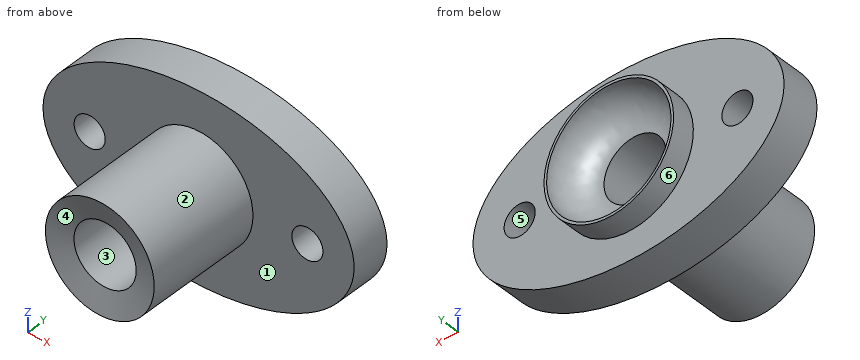
```python
from build123d import *

# Parameters (mm, degrees)
SHANK_SKETCH_42_R          = 21
SHANK_42_DEPTH             = 45
FLANGE_SKETCH_120X36_RX    = 60
FLANGE_SKETCH_120X36_RY    = 36
OVAL_FLANGE_120X36_DEPTH   = 15
SPIGOT_SKETCH_50_R         = 25
SPIGOT_50_DEPTH            = 9
MOUNTING_HOLES_SKETCH_R    = 6
MOUNTING_HOLES_2X_12_DEPTH = 19


with BuildPart() as part:
    # Shank Sketch Ø42 → Shank Ø42 (new body)
    with BuildSketch(Plane(origin=(0, 0, 0), x_dir=(1, 0, 0), z_dir=(0, 1, 0))):
        with Locations(Location((0, 0, 0), (0, 0, 90))):
            Circle(SHANK_SKETCH_42_R)
    extrude(amount=SHANK_42_DEPTH)

    # Flange Sketch 120x36 → Oval Flange 120x36 (add)
    with BuildSketch(Plane(origin=(0, 45, 0), x_dir=(1, 0, 0), z_dir=(0, 1, 0))):
        with Locations((0, 0)):
            Ellipse(FLANGE_SKETCH_120X36_RX, FLANGE_SKETCH_120X36_RY)
    extrude(amount=OVAL_FLANGE_120X36_DEPTH)

    # Spigot Sketch Ø50 → Spigot Ø50 (add)
    with BuildSketch(Plane(origin=(0, 60, 0), x_dir=(1, 0, 0), z_dir=(0, 1, 0))):
        with Locations(Location((0, 0, 0), (0, 0, 270))):
            Circle(SPIGOT_SKETCH_50_R)
    extrude(amount=SPIGOT_50_DEPTH)

    # Bore Profile Sketch → Bore and Seat Cut (revolve, cut)
    with BuildSketch(Plane.XY, mode=Mode.PRIVATE) as bore_and_seat_cut_sk:
        with BuildLine():
            Line((21, 0), (12, 2.411542732))
            Line((12, 2.411542732), (12, 57))
            ThreePointArc((12, 57), (20.485281374, 60.514718626), (24, 69))
            Line((24, 69), (0, 69))
            Line((0, 69), (0, 0))
            Line((0, 0), (21, 0))
        make_face()
    revolve(bore_and_seat_cut_sk.sketch.rotate(Axis((0, 0, 0), (0, 1, 0)), 90), axis=Axis((0, 0, 0), (0, 1, 0)), mode=Mode.SUBTRACT)

    # Mounting Holes Sketch → Mounting Holes 2xØ12 (cut)
    with BuildSketch(Plane(origin=(0, 60, 0), x_dir=(1, 0, 0), z_dir=(0, 1, 0))):
        with Locations(Location((-42, 0, 0), (0, 0, 270))):
            Circle(MOUNTING_HOLES_SKETCH_R)
        with Locations(Location((42, 0, 0), (0, 0, 270))):
            Circle(MOUNTING_HOLES_SKETCH_R)
    extrude(amount=-MOUNTING_HOLES_2X_12_DEPTH, mode=Mode.SUBTRACT)


solid = part.part
```
Work out the finished part from the listing and answer in its coordinate system (mm). Face numbers are marked on the shaded views. A direction names the side the tool comes from. Give positions to 0.01 mm unless a question says otherwise; leave off trailing zeros. Loops run counter-clockwise (first coordinate to the right, second up) from the corner with the lowest first, then second, coordinate; pieces in that order, holes last. Notation, with made-up numbers: (-24, -36) - (-6, -36) arc R27 cw to (-6, -4) - close; hole circle Ø1 at (40.5, 64.25). An arc over 180 degrees is marked (long way). One line per question, with ' | ' between items.
(1) The part is cut by section B-B (y = 30). Write down the section's boundary in (x, z), then the cut area to 3 significant figures.
Recorded:
outline: circle Ø42 at (0, 0); hole circle Ø24 at (0, 0) | area: 933 mm²
(2) A tool of negligible diameter and unlimited length cuts with its end or side. For the marked faces 5 and 6, from which of +Z, -Z, +X, -X, +Y, -Y can it reach the whole face along a straight path? Write none if from no direction.
Recorded:
face 5: +Y, -Y | face 6: +Y
(3) The mould has two halves that part along Z. Classify the marked faces 1, 2, 3 and 4: +Z half, -Z half, draft (parallel to the pull), parting line (faces both ways), or undercut.
Recorded:
face 1: draft | face 2: parting line | face 3: undercut | face 4: undercut
(4) Each of these flat-tipped pins is pushed along its axis until it touches: pin 1 Ø14 at (x, z) = (42, 0) entering from -Y; pin 2 Ø1 at (y, z) = (28.5, 0) entering from -X; pin 3 Ø7 at (x, z) = (-42, 0) entering from +Y; pin 4 Ø12 at (x, z) = (-8, 24) entering from -Y. Where does it stop, or does it pass through?
Recorded:
pin 1: stops at y = 45 | pin 2: stops at x = -21 | pin 3: passes through | pin 4: stops at y = 0
(5) The part is cut by section A-A (z = 0). Count the separate pieces of the cut face and the enclosed holes in it, then the cut area to 3 significant figures.
Recorded:
separate pieces: 4 | enclosed holes: 0 | area: 1,880 mm²
(6) Straight lines are drawn through the part: probe 1 along X at (y, z) = (54.5, 0); probe 2 along X at (y, z) = (13, 0); probe 3 along Y at (x, z) = (-35.5, -21.5). For each, find the intervals that lie inside material, in ascending order.
Recorded:
probe 1: x = -60 to -48, -36 to -12, 12 to 36, 48 to 60 | probe 2: x = -21 to -12, 12 to 21 | probe 3: y = 45 to 60
